CAD build for the part. Positions are in the model's coordinates, mm. Coordinates: 2 decimals unless noted, no trailing zeros. Loops run counter-clockwise (first coordinate to the right, second up) from the corner with the lowest first, then second, coordinate; pieces in that order, holes last. Notation, with made-up numbers: (13, 54.5) -> (55, 54.5) arc R34 cw to (55, 88.5) -> close; hole circle Ø6 at (41.5, -25). An arc over 180 degrees is marked (long way). Write each question's results on one line, items separated by ' | '.
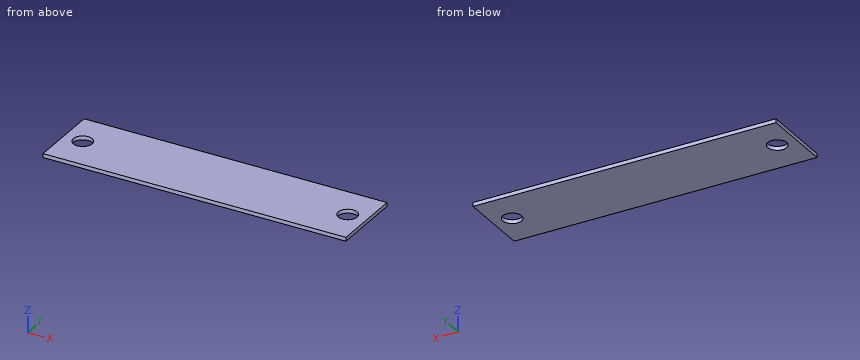
```python
from build123d import *

# Parameters (mm, degrees)
SKETCH_1_W            = 80
SKETCH_1_H            = 19
EXTRUDE_1_DEPTH       = 1
HOLE_WIZARD_5_0_5_1_D = 5


with BuildPart() as part:
    # 草图1 → 凸台-拉伸1 (new body)
    with BuildSketch(Plane.XY):
        with Locations((0, 9.5)):
            Rectangle(SKETCH_1_W, SKETCH_1_H)
    extrude(amount=EXTRUDE_1_DEPTH)

    # Ø5.0 (5) 直径孔1 (through all)
    with Locations(Plane.XY.offset(1)):
        with Locations((-35, 9.621851999), (35, 9.621851999)):
            Hole(HOLE_WIZARD_5_0_5_1_D / 2)


solid = part.part
```
Q1. Cut at B-B on y = 10.75. Write the cut outline in (x, z).
Results are:
outline: (-40, 0) -> (-37.23, 0) -> (-37.23, 1) -> (-40, 1) -> close; (-32.77, 0) -> (32.77, 0) -> (32.77, 1) -> (-32.77, 1) -> close; (37.23, 0) -> (40, 0) -> (40, 1) -> (37.23, 1) -> close
Q2. Drop a flat-ended pin along its axis: pin 1 (4.5 mm diameter, centred on x = 35, y = 9.62, fed in from -Z). Give the stop position or say it passes through.
Results are:
pin 1: through
Q3. Wall check: L1, parallel to X at y = 9.5, z = 0.8; L2, parallel to Y at x = 35, z = 0.55. Give the ranges that are in metal, low to high. Write a range as from..to.
Results are:
L1: -40..-37.5, -32.5..32.5, 37.5..40 | L2: 0..7.12, 12.12..19
Q4. Cut at C-C on z = 0.8. Write the cut outline in (x, y).
Results are:
outline: (-40, 0) -> (40, 0) -> (40, 19) -> (-40, 19) -> close; hole circle Ø5 at (-35, 9.62); hole circle Ø5 at (35, 9.62)
Q5. Cut at A-A on x = 35. Write the cut outline in (y, z).
Results are:
outline: (0, 0) -> (7.12, 0) -> (7.12, 1) -> (0, 1) -> close; (12.12, 0) -> (19, 0) -> (19, 1) -> (12.12, 1) -> close
